For this review, take the finished solid that the model builds, in its own axes (mm). Face numbers are marked on the shaded views. A direction names the side the tool comes from. Give positions to 0.01 mm unless a question says otherwise; leave off trailing zeros. Loops run counter-clockwise (first coordinate to the right, second up) from the corner with the lowest first, then second, coordinate; pieces in that order, holes last.
```python
from build123d import *
from build123d.topology import SkipClean

# Parameters (mm, degrees)
CLEVIS_LUG_1_SKETCH_R     = 28
CLEVIS_LUG_1_SKETCH_R_2   = 15
CLEVIS_LUG_1_56X_30_DEPTH = 26
CLEVIS_LUG_2_SKETCH_R     = 28
CLEVIS_LUG_2_SKETCH_R_2   = 15
CLEVIS_LUG_2_56X_30_DEPTH = 26
ARM_START                 = -16
ARM_BODY_DEPTH            = 16
ARM_EXTENSION_DEPTH       = 16
FORK_SLOT_SKETCH_W        = 16
FORK_SLOT_SKETCH_H        = 28
FORK_SLOT_CUT_DEPTH       = 32
PIVOT_BLOCK_SKETCH_W      = 39.579982786
PIVOT_BLOCK_SKETCH_H      = 40
PIVOT_BLOCK_DEPTH         = 48
TOP_PIVOT_BOSS_SKETCH_R   = 16
TOP_PIVOT_BOSS_SKETCH_R_2 = 8
TOP_PIVOT_BOSS_32_DEPTH   = 40
PIVOT_START               = -40
PIVOT_BORE_SKETCH_R       = 8
PIVOT_BORE_16_DEPTH       = 40
BOSS_GUSSET_DEPTH         = 5


with BuildPart() as part:
    # Clevis Lug 1 Sketch → Clevis Lug 1 Ø56xØ30 (new body)
    with BuildSketch(Plane(origin=(0, 0, 0), x_dir=(0, 0, -1), z_dir=(1, 0, 0))):
        with Locations(Location((0, 0, 0), (0, 0, 180))):
            Circle(CLEVIS_LUG_1_SKETCH_R)
        with Locations(Location((0, 0, 0), (0, 0, 180))):
            Circle(CLEVIS_LUG_1_SKETCH_R_2, mode=Mode.SUBTRACT)
    extrude(amount=CLEVIS_LUG_1_56X_30_DEPTH)



with BuildPart() as body_2:
    # Clevis Lug 2 Sketch → Clevis Lug 2 Ø56xØ30 (new body)
    with BuildSketch(Plane(origin=(-16, 0, 0), x_dir=(0, 0, -1), z_dir=(1, 0, 0))):
        with Locations(Location((0, 0, 0), (0, 0, 180))):
            Circle(CLEVIS_LUG_2_SKETCH_R)
        with Locations(Location((0, 0, 0), (0, 0, 180))):
            Circle(CLEVIS_LUG_2_SKETCH_R_2, mode=Mode.SUBTRACT)
    extrude(amount=-CLEVIS_LUG_2_56X_30_DEPTH)

    # Arm Profile Sketch → Arm Body (add)
    with BuildSketch(Plane(origin=(-16, 0, 0), x_dir=(0, 0, -1), z_dir=(1, 0, 0)).offset(ARM_START)):
        with BuildLine():
            Line((72, 28), (0, 28))
            ThreePointArc((0, 28), (19.798989873, 19.798989873), (28, 0))
            Line((28, 0), (30.92820323, 0))
            Line((30.92820323, 0), (30.92820323, 4))
            ThreePointArc((30.92820323, 4), (33.271348981, 9.656854249), (38.92820323, 12))
            Line((38.92820323, 12), (72, 12))
            Line((72, 12), (80, 12))
            ThreePointArc((80, 12), (86.92820323, 8), (86.92820323, 0))
            Line((86.92820323, 0), (114.92820323, 0))
            Line((114.92820323, 0), (114.92820323, 40))
            Line((114.92820323, 40), (78.92820323, 40))
            ThreePointArc((78.92820323, 40), (78.92820323, 32), (72, 28))
        make_face()
    extrude(amount=ARM_BODY_DEPTH)


with BuildPart() as part_1:
    with SkipClean():  # the faces are left unmerged after this step: merging them gives an invalid solid
        add(part.part)

        add(body_2.part)  # Arm Extension merges body 2
        # Arm Extension Sketch → Arm Extension (add, symmetric)
        with BuildSketch(Plane.ZY):
            with BuildLine():
                Line((0, 28), (-72, 28))
                ThreePointArc((-72, 28), (-78.92820323, 32), (-78.92820323, 40))
                Line((-78.92820323, 40), (-114.92820323, 40))
                Line((-114.92820323, 40), (-114.92820323, 0))
                Line((-114.92820323, 0), (-86.92820323, 0))
                ThreePointArc((-86.92820323, 0), (-86.92820323, 8), (-80, 12))
                Line((-80, 12), (-38.92820323, 12))
                ThreePointArc((-38.92820323, 12), (-33.271348981, 9.656854249), (-30.92820323, 4))
                Line((-30.92820323, 4), (-30.92820323, 0))
                Line((-30.92820323, 0), (-15, 0))
                ThreePointArc((-15, 0), (-10.606601718, 10.606601718), (0, 15))
                Line((0, 15), (0, 28))
            make_face()
        extrude(amount=ARM_EXTENSION_DEPTH, both=True)

    # Fork Slot Sketch → Fork Slot Cut (cut)
    with BuildSketch(Plane(origin=(0, 28, 0), x_dir=(1, 0, 0), z_dir=(0, 1, 0))):
        with Locations((-8, 14)):
            Rectangle(FORK_SLOT_SKETCH_W, FORK_SLOT_SKETCH_H)
    extrude(amount=-FORK_SLOT_CUT_DEPTH, mode=Mode.SUBTRACT)

    # Pivot Block Sketch → Pivot Block (add)
    with BuildSketch(Plane(origin=(16, 0, 0), x_dir=(0, 0, -1), z_dir=(1, 0, 0))):
        with Locations((115.138211837, 20)):
            Rectangle(PIVOT_BLOCK_SKETCH_W, PIVOT_BLOCK_SKETCH_H)
    extrude(amount=-PIVOT_BLOCK_DEPTH)

    # Top Pivot Boss Sketch → Top Pivot Boss Ø32 (add)
    with BuildSketch(Plane(origin=(0, 40, 0), x_dir=(1, 0, 0), z_dir=(0, 1, 0))):
        with Locations(Location((-8, 106.92820323, 0), (0, 0, 90))):
            Circle(TOP_PIVOT_BOSS_SKETCH_R)
        with Locations(Location((-8, 106.92820323, 0), (0, 0, 270))):
            Circle(TOP_PIVOT_BOSS_SKETCH_R_2, mode=Mode.SUBTRACT)
    extrude(amount=TOP_PIVOT_BOSS_32_DEPTH)

    # Pivot Bore Sketch → Pivot Bore Ø16 (cut)
    with BuildSketch(Plane(origin=(0, 40, 0), x_dir=(1, 0, 0), z_dir=(0, 1, 0)).offset(PIVOT_START)):
        with Locations(Location((-8, 106.92820323, 0), (0, 0, 270))):
            Circle(PIVOT_BORE_SKETCH_R)
    extrude(amount=PIVOT_BORE_16_DEPTH, mode=Mode.SUBTRACT)

    # Boss Gusset Sketch → Boss Gusset (add, symmetric)
    with BuildSketch(Plane(origin=(-8, 0, 0), x_dir=(0, 0, -1), z_dir=(1, 0, 0))):
        with BuildLine():
            Line((90.92820323, 80), (48, 28))
            Line((48, 28), (72, 28))
            ThreePointArc((72, 28), (78.92820323, 32), (78.92820323, 40))
            Line((78.92820323, 40), (93.443690624, 40))
            Line((93.443690624, 40), (93.443690624, 80))
            Line((93.443690624, 80), (90.92820323, 80))
        make_face()
    extrude(amount=BOSS_GUSSET_DEPTH, both=True)


solid = part_1.part
```
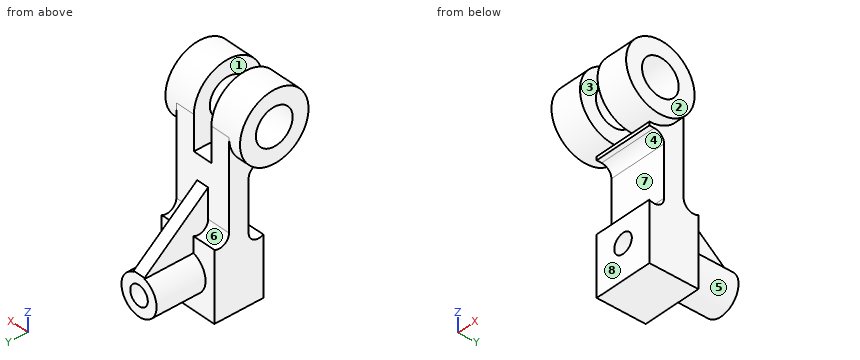
Item 1: Tool access review of the marked faces 5, 6, 7 and 8: name each direction out of +Z, -Z, +X, -X, +Y, -Y from which nothing blocks a thin tool from reaching the whole face with its end or side.
Answer:
face 5: +Y
face 6: +Z, -X
face 7: +X, -X, -Y
face 8: -Z, +X, -X, -Y
Item 2: Take a section at D-D on y = -5. Give the boundary of the cut face in (x, z).
Answer:
outline: (-42, -27.55) - (-16, -27.55) - (-16, -14.14) - (-42, -14.14) - close; (-42, 14.14) - (-16, 14.14) - (-16, 27.55) - (-42, 27.55) - close; (0, -27.55) - (26, -27.55) - (26, -14.14) - (0, -14.14) - close; (0, 14.14) - (26, 14.14) - (26, 27.55) - (0, 27.55) - close
Item 3: Take a section at C-C on x = -8. Give the boundary of the cut face in (y, z), and give its area (3 significant figures).
Answer:
outline: (0, -134.93) - (40, -134.93) - (40, -122.93) - (80, -122.93) - (80, -114.93) - (0, -114.93) - close; (0, -98.93) - (80, -98.93) - (80, -90.93) - (28, -48) - (28, -28) - (0, -28) - (0, -30.93) - (4, -30.93) arc R8 cw to (12, -38.93) - (12, -80) arc R8 cw to (0, -86.93) - close
area: 3,980 mm2
Item 4: For L1, parallel to Y at x = -28, z = 0; L2, parallel to X at y = 31, z = -126; L3, parallel to X at y = -21, z = 13, list the stretches that pass through material, from the lowest coordinate up.
Answer:
L1: y = -28 to -15, 15 to 28
L2: x = -32 to 16
L3: x = -42 to -16, 0 to 26
Item 5: Clearance check with flat-ended pins moving along their axes: pin 1 Ø24 at (x, z) = (0.5, -27.5) entering from +Y; pin 2 Ø13 at (y, z) = (42, -73.5) entering from +X; pin 3 Ø13 at (y, z) = (42.5, -61) entering from -X; pin 4 Ø24 at (y, z) = (0, 0) entering from +X. State where each tip first meets the part, or that it passes through.
Answer:
pin 1: stops at y = 28
pin 2: stops at x = 16
pin 3: stops at x = -13
pin 4: passes through
Item 6: The part is to be moulded in two halves that separate along X. For the marked faces 1, 2, 3 and 4, say which applies: released by +X, released by -X, zero draft, split by the parting line, or undercut.
Answer:
face 1: undercut
face 2: released by +X
face 3: undercut
face 4: zero draft
Item 7: Take a section at A-A on x = -30. Give the boundary of the cut face in (y, z).
Answer:
outline: (0, -134.93) - (40, -134.93) - (40, -78.93) arc R8 cw to (28, -72) - (28, 0) arc R28 ccw (long way) to (0, -28) - (0, -30.93) - (4, -30.93) arc R8 cw to (12, -38.93) - (12, -80) arc R8 cw to (0, -86.93) - close; hole circle Ø30 at (0, 0)
Item 8: Take a section at B-B on y = -21. Give the boundary of the cut face in (x, z), and give its area (3 significant figures).
Answer:
outline: (-42, -18.52) - (-16, -18.52) - (-16, 18.52) - (-42, 18.52) - close; (0, -18.52) - (26, -18.52) - (26, 18.52) - (0, 18.52) - close
area: 1,930 mm2
